from build123d import *

# Parameters (mm, degrees)
SKETCH1_W               = 60
SKETCH1_H               = 60
BOSS_EXTRUDE1_DEPTH     = 400
SKETCH2_W               = 50
SKETCH2_H               = 50
CUT_EXTRUDE1_DEPTH      = 5
SKETCH3_R               = 20
CUT_EXTRUDE2_DEPTH      = 20
SKETCH4_R               = 10
CUT_EXTRUDE3_DEPTH      = 15
FILLET1_R               = 3
CUT_EXTRUDE4_DEPTH      = 30
CUT_EXTRUDE4_DEPTH_BACK = 30
SKETCH5_R               = 4
SKETCH6_W               = 50
SKETCH6_H               = 50
CUT_EXTRUDE5_DEPTH      = 60
SKETCH7_R               = 25
CUT_EXTRUDE6_DEPTH      = 300
CUT_EXTRUDE7_DEPTH      = 30
CUT_EXTRUDE7_DEPTH_BACK = 30
SKETCH8_R               = 4
CUT_EXTRUDE9_DEPTH      = 30
CUT_EXTRUDE9_DEPTH_BACK = 30
SKETCH10_R              = 4
FILLET2_R               = 3
SKETCH11_R              = 2.5
CUT_EXTRUDE11_DEPTH     = 20


with BuildPart() as part:
    # Sketch1 → Boss-Extrude1 (new body)
    with BuildSketch(Plane(origin=(0, 0, 0), x_dir=(1, 0, 0), z_dir=(0, 1, 0))):
        Rectangle(SKETCH1_W, SKETCH1_H)
    extrude(amount=BOSS_EXTRUDE1_DEPTH)

    # Sketch2 → Cut-Extrude1 (cut)
    with BuildSketch(Plane(origin=(0, 400, 0), x_dir=(1, 0, 0), z_dir=(0, 1, 0))):
        Rectangle(SKETCH2_W, SKETCH2_H)
    extrude(amount=-CUT_EXTRUDE1_DEPTH, mode=Mode.SUBTRACT)

    # Sketch3 → Cut-Extrude2 (cut)
    with BuildSketch(Plane(origin=(0, 395, 0), x_dir=(1, 0, 0), z_dir=(0, 1, 0))):
        with Locations(Location((0, 0, 0), (0, 0, 270))):
            Circle(SKETCH3_R)
    extrude(amount=-CUT_EXTRUDE2_DEPTH, mode=Mode.SUBTRACT)

    # Sketch4 → Cut-Extrude3 (cut)
    with BuildSketch(Plane(origin=(0, 375, 0), x_dir=(1, 0, 0), z_dir=(0, 1, 0))):
        with Locations(Location((0, 0, 0), (0, 0, 270))):
            Circle(SKETCH4_R)
    extrude(amount=-CUT_EXTRUDE3_DEPTH, mode=Mode.SUBTRACT)

    # Fillet1
    fillet1_edges = [part.edges().sort_by_distance(p)[0] for p in [
        (-30, 200, -30),
        (-30, 200, 30),
        (30, 200, 30),
        (30, 200, -30),
    ]]
    fillet(fillet1_edges, radius=FILLET1_R)

    # Sketch5 → Cut-Extrude4 (cut, two sides: drawn at the far end of the back side and taken through both)
    with BuildSketch(Plane(origin=(0, 0, 0), x_dir=(0, 0, -1), z_dir=(1, 0, 0)).offset(-CUT_EXTRUDE4_DEPTH_BACK)):
        with Locations(Location((0, 385, 0), (0, 0, 180))):
            Circle(SKETCH5_R)
    extrude(amount=CUT_EXTRUDE4_DEPTH + CUT_EXTRUDE4_DEPTH_BACK, mode=Mode.SUBTRACT)

    # Sketch6 → Cut-Extrude5 (cut)
    with BuildSketch(Plane.XZ):
        Rectangle(SKETCH6_W, SKETCH6_H)
    extrude(amount=-CUT_EXTRUDE5_DEPTH, mode=Mode.SUBTRACT)

    # Sketch7 → Cut-Extrude6 (cut)
    with BuildSketch(Plane.XZ.offset(-60)):
        with Locations(Location((0, 0, 0), (0, 0, 270))):
            Circle(SKETCH7_R)
    extrude(amount=-CUT_EXTRUDE6_DEPTH, mode=Mode.SUBTRACT)

    # Sketch8 → Cut-Extrude7 (cut, two sides: drawn at the far end of the back side and taken through both)
    with BuildSketch(Plane(origin=(0, 0, 0), x_dir=(0, 0, -1), z_dir=(1, 0, 0)).offset(-CUT_EXTRUDE7_DEPTH_BACK)):
        with Locations(Location((0, 225, 0), (0, 0, 180))):
            Circle(SKETCH8_R)
    extrude(amount=CUT_EXTRUDE7_DEPTH + CUT_EXTRUDE7_DEPTH_BACK, mode=Mode.SUBTRACT)

    # Sketch10 → Cut-Extrude9 (cut, two sides: drawn at the far end of the back side and taken through both)
    with BuildSketch(Plane.XY.offset(-CUT_EXTRUDE9_DEPTH_BACK)):
        with Locations((-16, 40)):
            Circle(SKETCH10_R)
        with Locations((-16, 10)):
            Circle(SKETCH10_R)
        with Locations(Location((16, 10, 0), (0, 0, 180))):
            Circle(SKETCH10_R)
        with Locations(Location((16, 40, 0), (0, 0, 180))):
            Circle(SKETCH10_R)
    extrude(amount=CUT_EXTRUDE9_DEPTH + CUT_EXTRUDE9_DEPTH_BACK, mode=Mode.SUBTRACT)

    # Fillet2
    fillet2_edges = [part.edges().sort_by_distance(p)[0] for p in [
        (25, 397.5, -25),
        (25, 397.5, 25),
        (-25, 397.5, 25),
        (-25, 397.5, -25),
    ]]
    fillet(fillet2_edges, radius=FILLET2_R)

    # Sketch11 → Cut-Extrude11 (cut)
    with BuildSketch(Plane(origin=(0, 395, 0), x_dir=(1, 0, 0), z_dir=(0, 1, 0))):
        with Locations(Location((-19, 19, 0), (0, 0, 270))):
            Circle(SKETCH11_R)
        with Locations(Location((19, 19, 0), (0, 0, 270))):
            Circle(SKETCH11_R)
        with Locations(Location((-19, -19, 0), (0, 0, 270))):
            Circle(SKETCH11_R)
        with Locations(Location((19, -19, 0), (0, 0, 270))):
            Circle(SKETCH11_R)
    extrude(amount=-CUT_EXTRUDE11_DEPTH, mode=Mode.SUBTRACT)


solid = part.part
Build history of the part. All positions in model axes, mm. A direction names the side the tool comes from. Give positions to 0.01 mm unless a question says otherwise; leave off trailing zeros. Order: outer loops, then holes, each group sorted by start corner. A loop starts at its lowest first (then second) coordinate and runs counter-clockwise, first axis right, second up. Notation, with made-up numbers: M 51,42 L 95,42 A27 cw 95,71 Z; hole C 41.25,-31.5 d4. An arc over 180 degrees is marked long. Put each result on its own line as item: value.
Item 1: Which spindle directions (+Z, -Z, +X, -X, +Y, -Y) get a long thin tool onto all of the face, cutting with end or side? Do faces 1 (the face through (16.521, 36.034, 27.465)), 2 (the face through (-20, 60, -19)), 3 (the face through (-19.524, 385.14, -4.336)). Say none if no direction does.
Results are:
face 1: +Z, -Z
face 2: -Y
face 3: +Y
Item 2: Cut at B-B on y = 10. Write the cut outline in (x, z).
Results are:
outline: M -30,-27 A3 ccw -27,-30 L -20,-30 L -20,-25 L -25,-25 L -25,25 L -20,25 L -20,30 L -27,30 A3 ccw -30,27 Z; M -12,-30 L 12,-30 L 12,-25 L -12,-25 Z; M -12,25 L 12,25 L 12,30 L -12,30 Z; M 20,-30 L 27,-30 A3 ccw 30,-27 L 30,27 A3 ccw 27,30 L 20,30 L 20,25 L 25,25 L 25,-25 L 20,-25 Z
Item 3: Wall check: probe 1 along X at (y, z) = (10, 26.2); probe 2 along Y at (x, z) = (-16, 26.5); probe 3 along Z at (x, y) = (2, 249). Give the ranges that are in metal, low to high.
Results are:
probe 1: -30 to -20, -12 to 12, 20 to 30
probe 2: 0 to 6, 14 to 36, 44 to 400
probe 3: -30 to -24.92, 24.92 to 30
Item 4: Pull direction Y, two halves, no side cores. Call faces 4 (the face through (0, 30, -25)), 5 (the face through (-27, 0, 0)), 6 (the face through (-24.871, 388.549, 1.846)): +Y half, -Y half, draft (parallel to the pull), parting line (faces both ways), or undercut.
Results are:
face 4: draft
face 5: -Y half
face 6: undercut
Item 5: Drop flat-ended pins along their axis: pin 1 Ø15 at (x, z) = (-12.5, -5.5) entering from -Y; pin 2 Ø1.5 at (x, z) = (-18, -18) entering from +Y; pin 3 Ø10.5 at (x, y) = (-16, 10) entering from -Z; pin 4 Ø4 at (x, z) = (20, -18) entering from +Y. Give the stop position or say it passes through.
Results are:
pin 1: y = 360
pin 2: y = 375
pin 3: z = -30
pin 4: y = 395
Item 6: Cut at C-C on y = 82.5. Write the cut outline in (x, z), then the cut area to 3 significant figures.
Results are:
outline: M -30,-27 A3 ccw -27,-30 L 27,-30 A3 ccw 30,-27 L 30,27 A3 ccw 27,30 L -27,30 A3 ccw -30,27 Z; hole C 0,0 d50
area: 1,630 mm2
Item 7: Cut at A-A on y = 385. Write the cut outline in (x, z).
Results are:
outline: M -30,-27 A3 ccw -27,-30 L 27,-30 A3 ccw 30,-27 L 30,-4 L 19.6,-4 A20 cw -19.6,-4 L -30,-4 Z; M -30,4 L -19.6,4 A20 cw 19.6,4 L 30,4 L 30,27 A3 ccw 27,30 L -27,30 A3 ccw -30,27 Z; hole C -19,-19 d5; hole C -19,19 d5; hole C 19,-19 d5; hole C 19,19 d5
